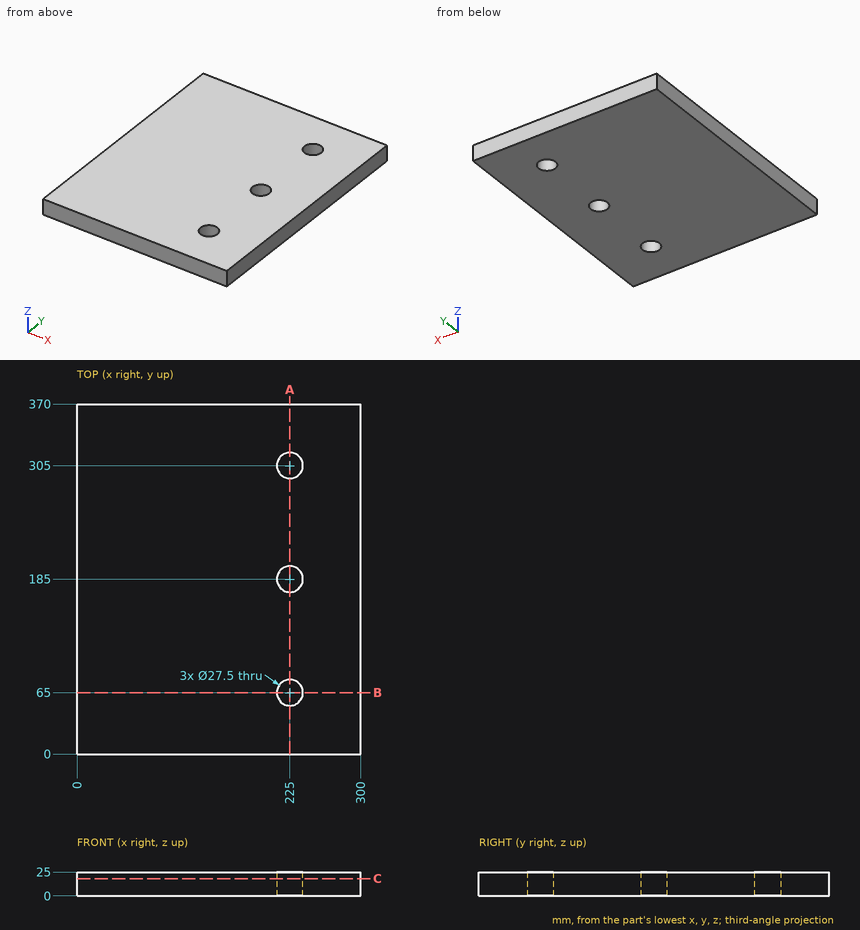
Input: dimensioned drawing with shaded views. Units: mm. Origin: part minimum x, y, z. Round coordinates to 2 decimals unless told otherwise and drop trailing zeros. Loops run counter-clockwise (first coordinate to the right, second up) from the corner with the lowest first, then second, coordinate; pieces in that order, holes last. Notation, with made-up numbers: (74, 41) -> (86, 41) arc R31 ccw to (86, 77) -> close; hole circle Ø5 at (58.5, 71). An arc over 180 degrees is marked (long way). One line per item, written item: value.
(1) Section C-C (z = 18). Return the cut outline in (x, y), plus the area to 3 significant figures.
Geometry check:
outline: (0, 0) -> (300, 0) -> (300, 370) -> (0, 370) -> close; hole circle Ø27.5 at (225, 65); hole circle Ø27.5 at (225, 185); hole circle Ø27.5 at (225, 305)
area: 109,000 mm2
(2) Material intervals for line 1 (Y direction, x = 225, z = 11.5); line 2 (X direction, y = 309.5, z = 7.5); line 3 (X direction, y = 67, z = 9.5), sorted ascending. Write a range as [from, to].
Geometry check:
line 1: [0, 51.25], [78.75, 171.25], [198.75, 291.25], [318.75, 370]
line 2: [0, 212.01], [237.99, 300]
line 3: [0, 211.4], [238.6, 300]
(3) Section B-B (y = 65). Return the cut outline in (x, z), plus the area to 3 significant figures.
Geometry check:
outline: (0, 0) -> (211.25, 0) -> (211.25, 25) -> (0, 25) -> close; (238.75, 0) -> (300, 0) -> (300, 25) -> (238.75, 25) -> close
area: 6,810 mm2
(4) Section A-A (x = 225). Return the cut outline in (y, z).
Geometry check:
outline: (0, 0) -> (51.25, 0) -> (51.25, 25) -> (0, 25) -> close; (78.75, 0) -> (171.25, 0) -> (171.25, 25) -> (78.75, 25) -> close; (198.75, 0) -> (291.25, 0) -> (291.25, 25) -> (198.75, 25) -> close; (318.75, 0) -> (370, 0) -> (370, 25) -> (318.75, 25) -> close
(5) Pin query (flat end, axial travel): pin 1 (25 mm diameter, centred on x = 225, y = 185, fed in from -Z). Return the tip coordinate at first contact, or that it passes through.
Geometry check:
pin 1: through
